Part model, mm, in its own coordinate system. A direction names the side the tool comes from. Coordinates: 2 decimals unless noted, no trailing zeros. Loops run counter-clockwise (first coordinate to the right, second up) from the corner with the lowest first, then second, coordinate; pieces in that order, holes last. Notation, with made-up numbers: (31, 64.5) - (78, 64.5) arc R18 cw to (78, 80.5) - close; hole circle Ø6 at (51, 49). An arc over 180 degrees is marked (long way). Answer as CSV lines item,"result".
from build123d import *

# Parameters (mm, degrees)
SKETCH_1_W               = 56
SKETCH_1_H               = 80
EXTRUDE_1_DEPTH          = 16
CUT_EXTRUDE_1_DEPTH      = 52.380930315
CUT_EXTRUDE_1_DEPTH_BACK = 52.380930315


with BuildPart() as part:
    # 草图1 → 凸台-拉伸1 (new body)
    with BuildSketch(Plane.XY):
        Rectangle(SKETCH_1_W, SKETCH_1_H)
    extrude(amount=EXTRUDE_1_DEPTH)

    # 草图2 → 切除-拉伸1 (cut, two sides: drawn at the far end of the back side and taken through both)
    with BuildSketch(Plane(origin=(0, 0, 0), x_dir=(-1, 0, 0), z_dir=(0, 0, -1)).offset(-CUT_EXTRUDE_1_DEPTH_BACK)):
        with BuildLine():
            Line((-12, 25.5), (8, 25.5))
            ThreePointArc((8, 25.5), (13.5, 20), (8, 14.5))
            Line((8, 14.5), (-12, 14.5))
            ThreePointArc((-12, 14.5), (-17.5, 20), (-12, 25.5))
        make_face()
        with BuildLine():
            Line((-12, -25.5), (8, -25.5))
            ThreePointArc((8, -25.5), (13.5, -20), (8, -14.5))
            Line((8, -14.5), (-12, -14.5))
            ThreePointArc((-12, -14.5), (-17.5, -20), (-12, -25.5))
        make_face()
    extrude(amount=CUT_EXTRUDE_1_DEPTH + CUT_EXTRUDE_1_DEPTH_BACK, mode=Mode.SUBTRACT)


solid = part.part
Q1. Two-plate mould, pull along X, no slides. Class faces 1 (the face through (17.5, -19.9, 8.1)), 2 (the face through (28, -1, 8)), 3 (the face through (0, 1, 16)): released by +X, released by -X, zero draft, split by the parting line, or undercut.
Results:
face 1,"undercut"
face 2,"released by +X"
face 3,"zero draft"
Q2. Which spindle directions (+Z, -Z, +X, -X, +Y, -Y) get a long thin tool onto all of the face, cutting with end or side? Do faces 4 (the face through (2, 14.5, 8)), 5 (the face through (0, 40, 8)). Say none if no direction does.
Results:
face 4,"+Z, -Z"
face 5,"+Z, -Z, +X, -X, +Y"
Q3. Saw through at C-C (z = 8.5). Give the cut face in (x, y), then the cut area to 3 significant figures.
Results:
outline,"(-28, -40) - (28, -40) - (28, 40) - (-28, 40) - close; hole (-8, -25.5) - (12, -25.5) arc R5.5 ccw to (12, -14.5) - (-8, -14.5) arc R5.5 ccw to start; hole (-8, 14.5) - (12, 14.5) arc R5.5 ccw to (12, 25.5) - (-8, 25.5) arc R5.5 ccw to start"
area,"3,850 mm^2"
Q4. Wall check: L1, parallel to Y at x = 4, z = 1.5; L2, parallel to Y at x = 15, z = 7.5; L3, parallel to X at y = 19, z = 12. Give the ranges that are in metal, low to high.
Results:
L1,"y = -40 to -25.5, -14.5 to 14.5, 25.5 to 40"
L2,"y = -40 to -24.61, -15.39 to 15.39, 24.61 to 40"
L3,"x = -28 to -13.41, 17.41 to 28"
Q5. Saw through at D-D (x = 2.5). Give the cut face in (y, z).
Results:
outline,"(-40, 0) - (-25.5, 0) - (-25.5, 16) - (-40, 16) - close; (-14.5, 0) - (14.5, 0) - (14.5, 16) - (-14.5, 16) - close; (25.5, 0) - (40, 0) - (40, 16) - (25.5, 16) - close"
Q6. Saw through at A-A (y = -20). Give the cut face in (x, z).
Results:
outline,"(-28, 0) - (-13.5, 0) - (-13.5, 16) - (-28, 16) - close; (17.5, 0) - (28, 0) - (28, 16) - (17.5, 16) - close"
Q7. Saw through at B-B (x = 15). Give the cut face in (y, z).
Results:
outline,"(-40, 0) - (-24.61, 0) - (-24.61, 16) - (-40, 16) - close; (-15.39, 0) - (15.39, 0) - (15.39, 16) - (-15.39, 16) - close; (24.61, 0) - (40, 0) - (40, 16) - (24.61, 16) - close"
